For this review, take the finished solid that the model builds, in its own axes (mm). A direction names the side the tool comes from. Give positions to 0.01 mm unless a question says otherwise; leave off trailing zeros. Order: outer loops, then holes, each group sorted by start corner. A loop starts at its lowest first (then second) coordinate and runs counter-clockwise, first axis right, second up. Notation, with made-up numbers: (19, 71) - (52, 71) arc R8 cw to (52, 79) - close; hole circle Ø4 at (44.5, 82). An arc over 180 degrees is marked (long way). Answer as a JSON object with one key per item and string values. Group by question number.
from build123d import *

# Parameters (mm, degrees)
BASE_WEB_DEPTH             = 60
UPPER_LUG_DEPTH            = 20
UPPER_LUG_BORE_SKETCH_R    = 15
UPPER_LUG_BORE_30_DEPTH    = 20
MOUNTING_FLANGE_DEPTH      = 20
FLANGE_BOSSES_SKETCH_R     = 20
FLANGE_BOSSES_SKETCH_R_2   = 10
FLANGE_BOSSES_DEPTH        = 30
LOWER_LUG_SKETCH_R         = 15
LOWER_LUG_DEPTH            = 40
FLANGE_START               = -40
FLANGE_BOSS_HOLES_SKETCH_R = 10
FLANGE_BOSS_HOLES_DEPTH    = 40


with BuildPart() as part:
    # Base Web Sketch → Base Web (new body)
    with BuildSketch(Plane.XY):
        Polygon((0, 0), (0, 60), (160, 60), (160, 0), (140, 0), (140, 40), (20, 40), (20, 0), align=None)
    extrude(amount=BASE_WEB_DEPTH)

    # Upper Lug Sketch → Upper Lug (add)
    with BuildSketch(Plane(origin=(0, 60, 0), x_dir=(1, 0, 0), z_dir=(0, 1, 0))):
        with BuildLine():
            Line((47, -93), (47, -60))
            Line((47, -60), (113, -60))
            Line((113, -60), (113, -93))
            ThreePointArc((113, -93), (80, -126), (47, -93))
        make_face()
    extrude(amount=-UPPER_LUG_DEPTH)

    # Upper Lug Bore Sketch → Upper Lug Bore Ø30 (cut)
    with BuildSketch(Plane(origin=(0, 60, 0), x_dir=(1, 0, 0), z_dir=(0, 1, 0))):
        with Locations(Location((80, -93, 0), (0, 0, 270))):
            Circle(UPPER_LUG_BORE_SKETCH_R)
    extrude(amount=-UPPER_LUG_BORE_30_DEPTH, mode=Mode.SUBTRACT)

    # Mounting Flange Sketch → Mounting Flange (add)
    with BuildSketch(Plane.XY):
        with BuildLine():
            Line((15, 60), (145, 60))
            ThreePointArc((145, 60), (130.857864376, 65.857864376), (125, 80))
            Line((125, 80), (125, 141.339700933))
            ThreePointArc((125, 141.339700933), (128.366825359, 152.445442752), (137.333750135, 159.812075252))
            Line((137.333750135, 159.812075252), (191.499374797, 182.29143852))
            ThreePointArc((191.499374797, 182.29143852), (209.981089089, 211.065033817), (189.504258609, 238.45468447))
            Line((189.504258609, 238.45468447), (125, 260))
            Line((125, 260), (35, 260))
            Line((35, 260), (-29.504258609, 238.45468447))
            ThreePointArc((-29.504258609, 238.45468447), (-49.981644615, 211.049278887), (-31.470247269, 182.279368197))
            Line((-31.470247269, 182.279368197), (22.646831513, 159.886795057))
            ThreePointArc((22.646831513, 159.886795057), (31.627336381, 152.520854718), (35, 141.406373855))
            Line((35, 141.406373855), (35, 80))
            ThreePointArc((35, 80), (29.142135624, 65.857864376), (15, 60))
        make_face()
    extrude(amount=MOUNTING_FLANGE_DEPTH)

    # Flange Bosses Sketch → Flange Bosses (add)
    # profile 1 of 2: a face of its own
    with BuildSketch(Plane.XY.offset(20)):
        with Locations((-20, 210)):
            Circle(FLANGE_BOSSES_SKETCH_R)
        with Locations((-20, 210)):
            Circle(FLANGE_BOSSES_SKETCH_R_2, mode=Mode.SUBTRACT)
    # profile 2 of 2: a face of its own
    with BuildSketch(Plane.XY.offset(20)):
        with Locations((180, 210)):
            Circle(FLANGE_BOSSES_SKETCH_R)
        with Locations((180, 210)):
            Circle(FLANGE_BOSSES_SKETCH_R_2, mode=Mode.SUBTRACT)
    extrude(amount=FLANGE_BOSSES_DEPTH)

    # Lower Lug Sketch → Lower Lug (add)
    with BuildSketch(Plane(origin=(0, 240, 0), x_dir=(1, 0, 0), z_dir=(0, 1, 0))):
        with BuildLine():
            Line((47, -93), (47, -30))
            ThreePointArc((47, -30), (49.928932188, -22.928932188), (57, -20))
            Line((57, -20), (103, -20))
            ThreePointArc((103, -20), (110.071067812, -22.928932188), (113, -30))
            Line((113, -30), (113, -93))
            ThreePointArc((113, -93), (80, -126), (47, -93))
        make_face()
        with Locations(Location((80, -93, 0), (0, 0, 270))):
            Circle(LOWER_LUG_SKETCH_R, mode=Mode.SUBTRACT)
    extrude(amount=-LOWER_LUG_DEPTH)

    # Flange Boss Holes Sketch → Flange Boss Holes (cut)
    with BuildSketch(Plane.XY.offset(20).offset(FLANGE_START)):
        with Locations(Location((-20, 210, 0), (0, 0, 180))):
            Circle(FLANGE_BOSS_HOLES_SKETCH_R)
        with Locations(Location((180, 210, 0), (0, 0, 180))):
            Circle(FLANGE_BOSS_HOLES_SKETCH_R)
    extrude(amount=FLANGE_BOSS_HOLES_DEPTH, mode=Mode.SUBTRACT)


solid = part.part
1) For faces 1 (the face through (164.037, 170.894, 9.86)), 2 (the face through (-25, 219, 50)), 3 (the face through (20, 20, 30)), 4 (the face through (80, 240, 72)), 5 (the face through (165.26, 223.52, 34.79)), list the 3-axis set-ups (+Z, -Z, +X, -X, +Y, -Y) from which the entire face can be reached by the end or side of a thin tool; tool diameter is ignored.
2) Consider section C-C (x = 80). Give the boundary of the cut face in (y, z).
3) Consider section D-D (x = 180). Give the boundary of the cut face in (y, z), plus the area to 3 significant figures.
4) Consider section B-B (z = 54). Give the boundary of the cut face in (x, y), plus the area to 3 significant figures.
5) For line 1 (X direction, y = 210, z = 7); line 2 (Y direction, x = 180, z = 29.25); line 3 (Y direction, x = 98, z = 51), list the stretches that pass through material, from the lowest coordinate up.
6) Mouldability with a two-part tool opening along Z and no side actions: class faces 6 (the face through (80.73, 50.14, 125.99)), 7 (the face through (66.69, 220.28, 99.92)), 8 (the face through (66.69, 50.14, 99.92)), 9 (the face through (140, 20, 30)) as released by +Z, released by -Z, zero draft, split by the parting line, or undercut.
7) Consider section A-A (z = 34). Give the boundary of the cut face in (x, y).
8) For pin 1 (10 mm diameter, centred on x = 85, z = 67, fed in from +Y); pin 2 (1 mm diameter, centred on y = 62, z = 65.5, fed in from +X); pin 3 (4 mm diameter, centred on x = -16.5, z = 24.5, fed in from -Y); pin 4 (6 mm diameter, centred on y = 52, z = 69.5, fed in from -X), all flat-tipped, find the tip position at first contact; note any pin that passes through.
Result set:
{
 "1": {"face 1": "+Z, -Z, +X", "face 2": "+Z, -X, +Y, -Y", "face 3": "+Z, -Z, -Y", "face 4": "+Z, +X, -X, +Y", "face 5": "+Z"},
 "2": {"outline": "(40, 0) - (260, 0) - (260, 20) - (240, 20) - (240, 78) - (200, 78) - (200, 20) - (60, 20) - (60, 78) - (40, 78) - close; (40, 108) - (60, 108) - (60, 126) - (40, 126) - close; (200, 108) - (240, 108) - (240, 126) - (200, 126) - close"},
 "3": {"outline": "(177.52, 0) - (200, 0) - (200, 50) - (190, 50) - (190, 20) - (177.52, 20) - close; (220, 0) - (241.63, 0) - (241.63, 20) - (230, 20) - (230, 50) - (220, 50) - close", "area": "1,480 mm2"},
 "4": {"outline": "(0, 0) - (20, 0) - (20, 40) - (140, 40) - (140, 0) - (160, 0) - (160, 60) - (0, 60) - close; (47, 200) - (113, 200) - (113, 240) - (47, 240) - close", "area": "7,440 mm2"},
 "5": {"line 1": "x = -50 to -30, -10 to 170, 190 to 210", "line 2": "y = 190 to 200, 220 to 230", "line 3": "y = 40 to 60, 200 to 240"},
 "6": {"face 6": "released by +Z", "face 7": "undercut", "face 8": "undercut", "face 9": "zero draft"},
 "7": {"outline": "circle Ø40 at (-20, 210); (0, 0) - (20, 0) - (20, 40) - (140, 40) - (140, 0) - (160, 0) - (160, 60) - (0, 60) - close; (47, 200) - (113, 200) - (113, 240) - (47, 240) - close; circle Ø40 at (180, 210); hole circle Ø20 at (-20, 210); hole circle Ø20 at (180, 210)"},
 "8": {"pin 1": "stops at y = 240", "pin 2": "passes through", "pin 3": "stops at y = 190.06", "pin 4": "stops at x = 47"}
}
